```python
from build123d import *

# Parameters (mm, degrees)
SKETCH1_W                                            = 150
SKETCH1_H                                            = 140
BOSS_EXTRUDE1_DEPTH                                  = 20
CHAMFER1_SIZE                                        = 5
SKETCH4_R                                            = 6
CUT_EXTRUDE1_DEPTH                                   = 3.2
SKETCH7_R                                            = 18
CUT_EXTRUDE2_DEPTH                                   = 105.522724802
M4_TAPPED_HOLE1_D                                    = 3.3
SKETCH14_W                                           = 60
SKETCH14_H                                           = 9
CUT_EXTRUDE5_DEPTH                                   = 50
M4_TAPPED_HOLE3_D                                    = 3.3
M4_TAPPED_HOLE3_DEPTH                                = 11.5
M4_TAPPED_HOLE3_TIP                                  = 0.991420021
FILLET1_R                                            = 5
HOLE_SIZE_PER_SOCKET_HEAD_CAP_SCREW_TYPE_D           = 6.6
HOLE_SIZE_PER_SOCKET_HEAD_CAP_SCREW_TYPE_CBORE_D     = 11
HOLE_SIZE_PER_SOCKET_HEAD_CAP_SCREW_TYPE_CBORE_DEPTH = 6.8
SKETCH23_W                                           = 121.756161874
SKETCH23_H                                           = 40
SKETCH23_H_2                                         = 40.700827196
CUT_EXTRUDE6_DEPTH                                   = 105.522724802
FILLET2_R                                            = 5
CHAMFER2_SIZE                                        = 5
HOLE_SIZE_PER_SOCKET_HEAD_CAP_SCREW_2_D              = 9
HOLE_SIZE_PER_SOCKET_HEAD_CAP_SCREW_2_CBORE_D        = 15
HOLE_SIZE_PER_SOCKET_HEAD_CAP_SCREW_2_CBORE_DEPTH    = 9
M6_TAPPED_HOLE1_D                                    = 5
M6_TAPPED_HOLE1_DEPTH                                = 17
M6_TAPPED_HOLE1_TIP                                  = 1.502151548
BLIND_DOWEL_HOLE1_SIZE_MM_D                          = 5
BLIND_DOWEL_HOLE1_SIZE_MM_DEPTH                      = 17
BLIND_DOWEL_HOLE1_SIZE_MM_TIP                        = 1.502151548
F_6_0_6_DIAMETER_HOLE1_D                             = 6
F_6_0_6_DIAMETER_HOLE1_DEPTH                         = 17
F_6_0_6_DIAMETER_HOLE1_TIP                           = 1.802581857


with BuildPart() as part:
    # Sketch1 → Boss-Extrude1 (new body)
    with BuildSketch(Plane(origin=(0, 0, 0), x_dir=(1, 0, 0), z_dir=(0, 1, 0))):
        Rectangle(SKETCH1_W, SKETCH1_H)
    extrude(amount=BOSS_EXTRUDE1_DEPTH)

    # Chamfer1
    chamfer1_edges = [part.edges().sort_by_distance(p)[0] for p in [
        (-75, 10, -70),
        (75, 10, -70),
        (75, 10, 70),
        (-75, 10, 70),
    ]]
    chamfer(chamfer1_edges, length=CHAMFER1_SIZE)

    # Sketch4 → Cut-Extrude1 (cut)
    with BuildSketch(Plane(origin=(0, 20, 0), x_dir=(1, 0, 0), z_dir=(0, 1, 0))):
        with Locations(Location((53, -51, 0), (0, 0, 270))):
            Circle(SKETCH4_R)
        with Locations(Location((53, 51, 0), (0, 0, 90))):
            Circle(SKETCH4_R)
    extrude(amount=-CUT_EXTRUDE1_DEPTH, mode=Mode.SUBTRACT)

    # Sketch7 → Cut-Extrude2 (cut, through all)
    with BuildSketch(Plane(origin=(0, 20, 0), x_dir=(1, 0, 0), z_dir=(0, 1, 0))):
        with Locations(Location((53, 0, 0), (0, 0, 270))):
            Circle(SKETCH7_R)
    extrude(amount=-CUT_EXTRUDE2_DEPTH, mode=Mode.SUBTRACT)

    # M4 Tapped Hole1 (through all)
    with Locations(Plane(origin=(0, 20, 0), x_dir=(-1, 0, 0), z_dir=(0, 1, 0))):
        with Locations((-68.5565, 15.5565), (-68.5565, -15.5565), (-37.4435, -15.5565), (-37.4435, 15.5565)):
            Hole(M4_TAPPED_HOLE1_D / 2)

    # Sketch14 → Cut-Extrude5 (cut)
    with BuildSketch(Plane(origin=(75, 0, 0), x_dir=(0, 0, -1), z_dir=(1, 0, 0))):
        with Locations((0, 4.5)):
            Rectangle(SKETCH14_W, SKETCH14_H)
    extrude(amount=-CUT_EXTRUDE5_DEPTH, mode=Mode.SUBTRACT)

    # M4 Tapped Hole3
    with Locations(Plane(origin=(75, 0, 0), x_dir=(0, 0, -1), z_dir=(1, 0, 0))):
        with Locations((-27.5, 14)):
            Hole(M4_TAPPED_HOLE3_D / 2, depth=M4_TAPPED_HOLE3_DEPTH)
            with Locations((0, 0, -(M4_TAPPED_HOLE3_DEPTH + M4_TAPPED_HOLE3_TIP / 2))):  # 118° drill point
                Cone(0, M4_TAPPED_HOLE3_D / 2, M4_TAPPED_HOLE3_TIP, mode=Mode.SUBTRACT)

    # Fillet1
    fillet1_edges = [part.edges().sort_by_distance(p)[0] for p in [
        (25, 4.5, 30),
        (25, 4.5, -30),
    ]]
    fillet(fillet1_edges, radius=FILLET1_R)

    # Hole size per socket head cap screw type (through all)
    with Locations(Plane(origin=(0, 0, 0), x_dir=(-1, 0, 0), z_dir=(0, -1, 0))):
        with Locations((-53, -51), (-53, 51)):
            CounterBoreHole(HOLE_SIZE_PER_SOCKET_HEAD_CAP_SCREW_TYPE_D / 2, HOLE_SIZE_PER_SOCKET_HEAD_CAP_SCREW_TYPE_CBORE_D / 2, HOLE_SIZE_PER_SOCKET_HEAD_CAP_SCREW_TYPE_CBORE_DEPTH)

    # Sketch23 → Cut-Extrude6 (cut, through all)
    with BuildSketch(Plane(origin=(0, 20, 0), x_dir=(1, 0, 0), z_dir=(0, 1, 0))):
        with Locations((-55.878080937, 60)):
            Rectangle(SKETCH23_W, SKETCH23_H)
        with Locations((-55.878080937, -60.350413598)):
            Rectangle(SKETCH23_W, SKETCH23_H_2)
    extrude(amount=-CUT_EXTRUDE6_DEPTH, mode=Mode.SUBTRACT)

    # Fillet2
    fillet2_edges = [part.edges().sort_by_distance(p)[0] for p in [
        (5, 10, -40),
        (5, 10, 40),
    ]]
    fillet(fillet2_edges, radius=FILLET2_R)

    # Chamfer2
    chamfer2_edges = [part.edges().sort_by_distance(p)[0] for p in [
        (5, 10, -70),
        (-75, 10, -40),
        (5, 10, 70),
        (-75, 10, 40),
    ]]
    chamfer(chamfer2_edges, length=CHAMFER2_SIZE)

    # Hole size per socket head cap screw  2 (through all)
    with Locations(Plane(origin=(0, 20, 0), x_dir=(1, 0, 0), z_dir=(0, 1, 0))):
        with Locations((25, 50), (25, -50), (-55, 20), (-55, -20)):
            CounterBoreHole(HOLE_SIZE_PER_SOCKET_HEAD_CAP_SCREW_2_D / 2, HOLE_SIZE_PER_SOCKET_HEAD_CAP_SCREW_2_CBORE_D / 2, HOLE_SIZE_PER_SOCKET_HEAD_CAP_SCREW_2_CBORE_DEPTH)

    # M6 Tapped Hole1
    with Locations(Plane(origin=(0, 20, 0), x_dir=(1, 0, 0), z_dir=(0, 1, 0))):
        with Locations((-9, 30.5), (-9, -30.5)):
            Hole(M6_TAPPED_HOLE1_D / 2, depth=M6_TAPPED_HOLE1_DEPTH)
            with Locations((0, 0, -(M6_TAPPED_HOLE1_DEPTH + M6_TAPPED_HOLE1_TIP / 2))):  # 118° drill point
                Cone(0, M6_TAPPED_HOLE1_D / 2, M6_TAPPED_HOLE1_TIP, mode=Mode.SUBTRACT)

    # Blind dowel hole1, size mm
    with Locations(Plane(origin=(0, 20, 0), x_dir=(-1, 0, 0), z_dir=(0, 1, 0))):
        with Locations((9, -15), (9, 15)):
            Hole(BLIND_DOWEL_HOLE1_SIZE_MM_D / 2, depth=BLIND_DOWEL_HOLE1_SIZE_MM_DEPTH)
            with Locations((0, 0, -(BLIND_DOWEL_HOLE1_SIZE_MM_DEPTH + BLIND_DOWEL_HOLE1_SIZE_MM_TIP / 2))):  # 118° drill point
                Cone(0, BLIND_DOWEL_HOLE1_SIZE_MM_D / 2, BLIND_DOWEL_HOLE1_SIZE_MM_TIP, mode=Mode.SUBTRACT)

    # Ø6.0 (6) Diameter Hole1
    with Locations(Plane(origin=(0, 0, 0), x_dir=(-1, 0, 0), z_dir=(0, -1, 0))):
        with Locations((55, 0), (-15, 0)):
            Hole(F_6_0_6_DIAMETER_HOLE1_D / 2, depth=F_6_0_6_DIAMETER_HOLE1_DEPTH)
            with Locations((0, 0, -(F_6_0_6_DIAMETER_HOLE1_DEPTH + F_6_0_6_DIAMETER_HOLE1_TIP / 2))):  # 118° drill point
                Cone(0, F_6_0_6_DIAMETER_HOLE1_D / 2, F_6_0_6_DIAMETER_HOLE1_TIP, mode=Mode.SUBTRACT)


solid = part.part
```
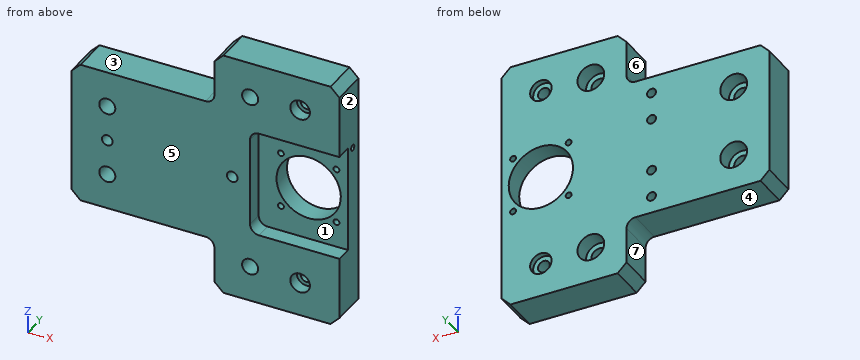
Model file for the job. Use its own axes, mm. Face numbers are marked on the shaded views. A direction names the side the tool comes from. Coordinates: 2 decimals unless noted, no trailing zeros. Loops run counter-clockwise (first coordinate to the right, second up) from the corner with the lowest first, then second, coordinate; pieces in that order, holes last. Notation, with made-up numbers: (76.25, -36) - (80.25, -36) arc R9 ccw to (80.25, -32) - close; hole circle Ø7 at (89, 87). An arc over 180 degrees is marked (long way). Write item = value, one per line. Start each with the question number.
Item 1: Drop flat-ended pins along their axis: pin 1 Ø6 at (x, y) = (-19.5, 11.5) entering from -Z; pin 2 Ø2.5 at (x, z) = (68.56, -15.56) entering from +Y; pin 3 Ø6 at (x, z) = (-9, -15) entering from +Y; pin 4 Ø12 at (y, z) = (2, -47) entering from -X. Give the stop position or say it passes through.
Item 2: Saw through at A-A, the plane z = -7.5. List the corners of the cut face in (x, y).
Item 3: Wall check: probe 1 along Z at (x, y) = (-55, 3.5); probe 2 along Z at (x, y) = (36, 3.5); probe 3 along Z at (x, y) = (53, 2.25). Give the ranges that are in metal, low to high. Write a range as [from, to].
Item 4: 3-axis set-ups, long thin cutter, end or side, ignore diameter. For the marked faces 5, 6 and 7: which of +Z, -Z, +X, -X, +Y, -Y reach the whole face in a straight line?
Item 5: Pull direction Z, two halves, no side cores. Call the marked faces 1, 2, 3 and 4: +Z half, -Z half, draft (parallel to the pull), parting line (faces both ways), or undercut.
Item 6: Saw through at B-B, the plane x = 53. State how many separate pieces and enclosed holes the cut face has, then the cut area to 3 significant figures.
Answers:
q1.pin_1 = -40
q1.pin_2 = through
q1.pin_3 = 20
q1.pin_4 = 3
q2.outline = (-75, 0) - (25, 0) - (25, 9) - (36.64, 9) - (36.64, 20) - (-75, 20) - close; (69.36, 9) - (75, 9) - (75, 20) - (69.36, 20) - close
q3.probe_1 = [-40, -24.5], [-15.5, -3], [3, 15.5], [24.5, 40]
q3.probe_2 = [-70, -30], [30, 70]
q3.probe_3 = [-70, -56.5], [-45.5, -30], [30, 45.5], [56.5, 70]
q4.face_5 = +Z, -Z, +X, -X, -Y
q4.face_6 = +Z, -X, +Y, -Y
q4.face_7 = -Z, -X, +Y, -Y
q5.face_1 = undercut
q5.face_2 = draft
q5.face_3 = +Z half
q5.face_4 = -Z half
q6.separate_pieces = 4
q6.enclosed_holes = 0
q6.area = 1,510 mm2
